```python
from build123d import *

# Parameters (mm, degrees)
SKETCH_1_W                                        = 33
SKETCH_1_H                                        = 60
BOSS_EXTRUDE_1_DEPTH                              = 8
SKETCH_2_W                                        = 33
SKETCH_2_H                                        = 25
BOSS_EXTRUDE_2_DEPTH                              = 18
M3_HEX_SOCKET_CAP_SCREW_COUNTERBORE_1_D           = 3.4
M3_HEX_SOCKET_CAP_SCREW_COUNTERBORE_1_CBORE_D     = 6.5
M3_HEX_SOCKET_CAP_SCREW_COUNTERBORE_1_CBORE_DEPTH = 3
LINEAR_PATTERN_1_COUNT                            = 2
LINEAR_PATTERN_1_PITCH                            = 23
LINEAR_PATTERN_1_COUNT_DIR2                       = 2
LINEAR_PATTERN_1_PITCH_DIR2                       = 25
LINEAR_PATTERN_2_COUNT                            = 2
LINEAR_PATTERN_2_PITCH                            = 10
SKETCH_9_W                                        = 33
SKETCH_9_H                                        = 5
CUT_EXTRUDE_1_DEPTH                               = 18
F_3_0_3_HOLE_1_D                                  = 3
LINEAR_PATTERN_3_COUNT                            = 2
LINEAR_PATTERN_3_PITCH                            = 25
LINEAR_PATTERN_4_COUNT                            = 2
LINEAR_PATTERN_4_PITCH                            = 16


with BuildPart() as part:
    # Sketch 1 → Boss-Extrude 1 (new body)
    with BuildSketch(Plane(origin=(0, 0, 0), x_dir=(0, 0, -1), z_dir=(1, 0, 0))):
        Rectangle(SKETCH_1_W, SKETCH_1_H)
    extrude(amount=BOSS_EXTRUDE_1_DEPTH)

    # Sketch 2 → Boss-Extrude 2 (add)
    with BuildSketch(Plane.ZY):
        with Locations((0, -17.5)):
            Rectangle(SKETCH_2_W, SKETCH_2_H)
    extrude(amount=BOSS_EXTRUDE_2_DEPTH)

    # M3 Hex Socket Cap Screw Counterbore 1 (through all)
    with Locations(Plane.ZY):
        with Locations((-11.5, 25)):
            m3_hex_socket_cap_screw_counterbore_1 = CounterBoreHole(M3_HEX_SOCKET_CAP_SCREW_COUNTERBORE_1_D / 2, M3_HEX_SOCKET_CAP_SCREW_COUNTERBORE_1_CBORE_D / 2, M3_HEX_SOCKET_CAP_SCREW_COUNTERBORE_1_CBORE_DEPTH)

    # Linear Pattern 1: M3 Hex Socket Cap Screw Counterbore 1 2 × 2
    with Locations(*[(0, -j * LINEAR_PATTERN_1_PITCH_DIR2, i * LINEAR_PATTERN_1_PITCH) for i in range(LINEAR_PATTERN_1_COUNT) for j in range(LINEAR_PATTERN_1_COUNT_DIR2) if (i, j) != (0, 0)]):
        add(m3_hex_socket_cap_screw_counterbore_1, mode=Mode.SUBTRACT)

    # Sketch 7 → M4 Tapped Hole 2 (revolve, cut)
    with BuildSketch(Plane(origin=(-18, -25, 0), x_dir=(0, 0, 1), z_dir=(0, 1, 0))):
        Polygon((0, 0), (0, 11.091420021), (1.65, 10.1), (1.65, 0), align=None)
    m4_tapped_hole_2 = revolve(axis=Axis((-24.35, -25, 0), (1, 0, 0)), mode=Mode.SUBTRACT)

    # Linear Pattern 2: M4 Tapped Hole 2 ×2
    with Locations(*[(0, i * LINEAR_PATTERN_2_PITCH, 0) for i in range(1, LINEAR_PATTERN_2_COUNT)]):
        add(m4_tapped_hole_2, mode=Mode.SUBTRACT)

    # Sketch 9 → Cut-Extrude 1 (cut)
    with BuildSketch(Plane.ZY.offset(18)):
        with Locations((0, -7.5)):
            Rectangle(SKETCH_9_W, SKETCH_9_H)
    extrude(amount=-CUT_EXTRUDE_1_DEPTH, mode=Mode.SUBTRACT)

    # Ø3.0 (3) Hole 1 (through all)
    with Locations(Plane.ZY):
        with Locations((11.5, 20)):
            f_3_0_3_hole_1 = Hole(F_3_0_3_HOLE_1_D / 2)

    # Linear Pattern 3: Ø3.0 (3) Hole 1 ×2
    with Locations(*[(0, -i * LINEAR_PATTERN_3_PITCH, 0) for i in range(1, LINEAR_PATTERN_3_COUNT)]):
        add(f_3_0_3_hole_1, mode=Mode.SUBTRACT)

    # Sketch 12 → Ø4.0 (4) Hole 1 (revolve, cut)
    with BuildSketch(Plane(origin=(-18, -20, -8), x_dir=(0, 0, 1), z_dir=(0, 1, 0))):
        Polygon((0, 0), (0, 11.201721238), (2, 10), (2, 0), align=None)
    f_4_0_4_hole_1 = revolve(axis=Axis((-24.35, -20, -8), (1, 0, 0)), mode=Mode.SUBTRACT)

    # Linear Pattern 4: Ø4.0 (4) Hole 1 ×2
    with Locations(*[(0, 0, i * LINEAR_PATTERN_4_PITCH) for i in range(1, LINEAR_PATTERN_4_COUNT)]):
        add(f_4_0_4_hole_1, mode=Mode.SUBTRACT)


solid = part.part
```
The model under review builds one solid part; all positions refer to its coordinate system, in mm. A direction names the side the tool comes from. Give positions to 0.01 mm unless a question says otherwise; leave off trailing zeros. Write each loop counter-clockwise with the first axis right and the second up, starting at its lowest first coordinate (ties: lowest second). Pieces come first, ordered by that corner, then holes. Notation, with made-up numbers: (57.5, 46) -> (113.5, 46) arc R31 cw to (113.5, 85) -> close; hole circle Ø2 at (69, -17). An arc over 180 degrees is marked (long way). Answer in a Markdown table with one row per item.
1) Mouldability with a two-part tool opening along Y and no side actions: class faces 1 (the cylindrical face through (-13.02, -16.39, 0.89)), 2 (the flat face through (8, 0, 0)) as +Y half, -Y half, draft (parallel to the pull), parting line (faces both ways), or undercut.
Worked answers:
| item | result |
|---|---|
| face 1 | undercut |
| face 2 | draft |
2) Add section D-D on z = 11.5. Count the separate pieces of the cut face and the enclosed holes in it, plus the area to 3 significant figures.
Worked answers:
| item | result |
|---|---|
| separate pieces | 5 |
| enclosed holes | 0 |
| area | 719 mm² |
3) Add section B-B on x = 1.5. State the section outline as (y, z) points.
Worked answers:
| item | result |
|---|---|
| outline | (-30, -16.5) -> (30, -16.5) -> (30, 16.5) -> (-30, 16.5) -> close; hole circle Ø3 at (-5, 11.5); hole circle Ø6.5 at (0, -11.5); hole circle Ø6.5 at (0, 11.5); hole circle Ø3 at (20, 11.5); hole circle Ø6.5 at (25, -11.5); hole circle Ø6.5 at (25, 11.5) |
4) Add section C-C on z = -11.5. State the section outline as (x, y) points.
Worked answers:
| item | result |
|---|---|
| outline | (-18, -30) -> (8, -30) -> (8, -1.7) -> (3, -1.7) -> (3, -3.25) -> (0, -3.25) -> (0, -10) -> (-18, -10) -> close; (0, 3.25) -> (3, 3.25) -> (3, 1.7) -> (8, 1.7) -> (8, 23.3) -> (3, 23.3) -> (3, 21.75) -> (0, 21.75) -> close; (0, 28.25) -> (3, 28.25) -> (3, 26.7) -> (8, 26.7) -> (8, 30) -> (0, 30) -> close |
5) Clearance check with flat-ended pins moving along their axes: P1, Ø3, axis at y = -1, z = -13, coming from the -X side; P2, Ø2.5, axis at y = 0, z = -11.5, coming from the +X side; P3, Ø5.5, axis at x = -6.5, z = -1, coming from the +Y side. State where each tip first meets the part, or that it passes through.
Worked answers:
| item | result |
|---|---|
| P1 | x = 0 |
| P2 | through |
| P3 | y = -10 |
6) Add section A-A on y = 25. State the section outline as (x, z) points, plus the area to 3 significant figures.
Worked answers:
| item | result |
|---|---|
| outline | (0, -16.5) -> (8, -16.5) -> (8, -13.2) -> (3, -13.2) -> (3, -14.75) -> (0, -14.75) -> close; (0, -8.25) -> (3, -8.25) -> (3, -9.8) -> (8, -9.8) -> (8, 9.8) -> (3, 9.8) -> (3, 8.25) -> (0, 8.25) -> close; (0, 14.75) -> (3, 14.75) -> (3, 13.2) -> (8, 13.2) -> (8, 16.5) -> (0, 16.5) -> close |
| area | 191 mm² |
7) Tool access review of faces 3 (the flat face through (0, 10, 0)), 4 (the cylindrical face through (5.535, 26.433, 10.586)), 5 (the cylindrical face through (1.479, 0.143, -14.747)): name each direction out of +Z, -Z, +X, -X, +Y, -Y from which nothing blocks a thin tool from reaching the whole face with its end or side.
Worked answers:
| item | result |
|---|---|
| face 3 | +Z, -Z, -X, +Y |
| face 4 | +X, -X |
| face 5 | -X |
8) For L1, parallel to Y at x = 6.4, z = -11.5; L2, parallel to Z at x = 1.75, y = 23; L3, parallel to X at y = -0.5, z = -1.5, list the stretches that pass through material, from the lowest coordinate up. Write a range as [from, to].
Worked answers:
| item | result |
|---|---|
| L1 | [-30, -1.7], [1.7, 23.3], [26.7, 30] |
| L2 | [-16.5, -14.06], [-8.94, 8.94], [14.06, 16.5] |
| L3 | [0, 8] |
